The figure shows three views and two pictorial views of one solid part (mm, origin at its lowest corner). Answer the questions. A direction names the side the tool comes from. Round coordinates to 2 decimals unless told otherwise and drop trailing zeros. Order: outer loops, then holes, each group sorted by start corner. A loop starts at its lowest first (then second) coordinate and runs counter-clockwise, first axis right, second up. Notation, with made-up numbers: (63, 62.5) - (113, 62.5) arc R11 cw to (113, 82.5) - close; hole circle Ø11 at (20.5, 56). An arc over 180 degrees is marked (long way). Use CSV: the item, a comma, the result in double quotes.
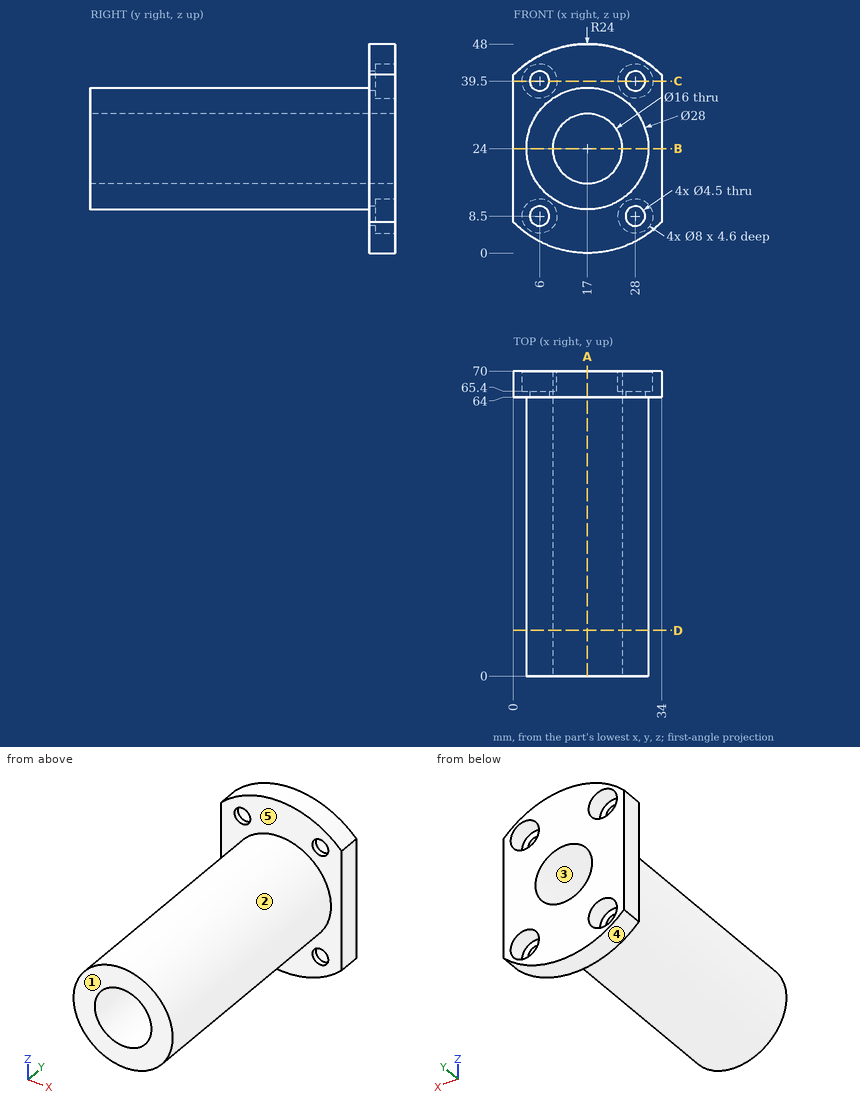
(1) The mould has two halves that part along X. Classify the marked faces 3, 4 and 5: released by +X, released by -X, zero draft, split by the parting line, or undercut.
Findings below:
face 3,"undercut"
face 4,"split by the parting line"
face 5,"zero draft"
(2) Find section A-A (x = 17). Determine the outline of the cut face in (y, z), and give its area (3 significant figures).
Findings below:
outline,"(0, 10) - (64, 10) - (64, 0) - (70, 0) - (70, 16) - (0, 16) - close; (0, 32) - (70, 32) - (70, 48) - (64, 48) - (64, 38) - (0, 38) - close"
area,"960 mm²"
(3) For the marked faces 1 and 2, determine the directions among +Z, -Z, +X, -X, +Y, -Y from which every point of the face is accessible in a straight line to the end or side of a thin tool.
Findings below:
face 1,"+Z, -Z, +X, -X, -Y"
face 2,"-Y"
(4) Each of these flat-tipped pins is pushed along its axis until it touches: pin 1 (2 mm diameter, centred on y = 45, z = 33.5, fed in from -X); pin 2 (10.5 mm diameter, centred on x = 6, z = 39.5, fed in from -Y); pin 3 (6 mm diameter, centred on y = 25, z = 32.5, fed in from +X); pin 4 (7 mm diameter, centred on x = 28, z = 39.5, fed in from -Y). Where does it stop, or does it pass through?
Findings below:
pin 1,"stops at x = 5.88"
pin 2,"stops at y = 0"
pin 3,"stops at x = 29.87"
pin 4,"stops at y = 64"
(5) Find the intervals of material crossed by L1, parallel to Z at x = 28, y = 67; L2, parallel to Z at x = 28, y = 65.15; L3, parallel to Z at x = 22.5, y = 12.5, in increasing order. Write a range as from..to.
Findings below:
L1,"z = 2.67..4.5, 12.5..35.5, 43.5..45.33"
L2,"z = 2.67..6.25, 10.75..37.25, 41.75..45.33"
L3,"z = 11.13..18.19, 29.81..36.87"
(6) Find section D-D (y = 10.5). Determine the outline of the cut face in (x, z).
Findings below:
outline,"circle Ø28 at (17, 24); hole circle Ø16 at (17, 24)"
(7) Find section C-C (z = 39.5). Determine the outline of the cut face in (x, y), and give its area (3 significant figures).
Findings below:
outline,"(0, 64) - (3.75, 64) - (3.75, 65.4) - (2, 65.4) - (2, 70) - (0, 70) - close; (8.25, 64) - (25.75, 64) - (25.75, 65.4) - (24, 65.4) - (24, 70) - (10, 70) - (10, 65.4) - (8.25, 65.4) - close; (30.25, 64) - (34, 64) - (34, 70) - (32, 70) - (32, 65.4) - (30.25, 65.4) - close"
area,"118 mm²"
(8) Find section B-B (z = 24). Determine the outline of the cut face in (x, y).
Findings below:
outline,"(0, 64) - (3, 64) - (3, 0) - (9, 0) - (9, 70) - (0, 70) - close; (25, 0) - (31, 0) - (31, 64) - (34, 64) - (34, 70) - (25, 70) - close"
